Design review of the part built by this model. Coordinates are the model's own, in mm. A direction names the side the tool comes from. Coordinates: 2 decimals unless noted, no trailing zeros. Order: outer loops, then holes, each group sorted by start corner. A loop starts at its lowest first (then second) coordinate and runs counter-clockwise, first axis right, second up. Notation, with made-up numbers: (69, -19) -> (116, -19) arc R30 cw to (116, 11) -> close; hole circle Ø6 at (-26.75, 38.25). An arc over 180 degrees is marked (long way). Write item = value, one per line.
```python
from build123d import *

# Parameters (mm, degrees)
BASE_EXTRUDE_DEPTH = 3.5
SKETCH4_W          = 0.5
SKETCH4_H          = 10.618802154
CHAMFER_2_SIZE     = 0.64
FILLET_2_R         = 0.2


with BuildPart() as part:
    # Sketch1 → Base-Extrude (new body)
    with BuildSketch(Plane(origin=(0, 0, 0), x_dir=(0, 0, -1), z_dir=(1, 0, 0))):
        Polygon((4, 2.309401077), (4, -2.309401077), (0, -4.618802154), (-4, -2.309401077), (-4, 2.309401077), (0, 4.618802154), align=None)
    extrude(amount=BASE_EXTRUDE_DEPTH)

    # Sketch2 → Boss-Revolve1 (revolve)
    with BuildSketch(Plane.XY, mode=Mode.PRIVATE) as boss_revolve1_sk:
        Polygon((0, 0), (13.5, 0), (13.5, 1.8072), (13.5, 2.5), (0, 2.5), align=None)
    revolve(boss_revolve1_sk.sketch.rotate(Axis((0, 0, 0), (1, 0, 0)), 90), axis=Axis((0, 0, 0), (1, 0, 0)))

    # Sketch3 → Cut-Revolve1 (revolve, cut)
    with BuildSketch(Plane.XY):
        Polygon((0, 4), (3.244016936, 9.618802154), (3.244016936, 14.618802154), (-10, 14.618802154), (-10, 4), align=None)
    revolve(axis=Axis((0, 0, 0), (1, 0, 0)), mode=Mode.SUBTRACT)

    # Sketch5 → Cut-Revolve2 (revolve, cut)
    with BuildSketch(Plane.XY):
        Polygon((3.5, 4), (0.255983064, 9.618802154), (0.255983064, 14.618802154), (10.255983064, 14.618802154), (10.255983064, 4), align=None)
    revolve(axis=Axis((0, 0, 0), (1, 0, 0)), mode=Mode.SUBTRACT)

    # Sketch4 → Cut-Revolve3 (revolve, cut)
    with BuildSketch(Plane.XY, mode=Mode.PRIVATE) as cut_revolve3_sk:
        with Locations((3.25, 9.309401077)):
            Rectangle(SKETCH4_W, SKETCH4_H)
    revolve(cut_revolve3_sk.sketch.rotate(Axis((0, 0, 0), (1, 0, 0)), 270), axis=Axis((0, 0, 0), (1, 0, 0)), mode=Mode.SUBTRACT)

    # Chamfer 2
    chamfer_2_edges = [part.edges().sort_by_distance(p)[0] for p in [
        (13.5, 0, -2.5),
    ]]
    chamfer(chamfer_2_edges, length=CHAMFER_2_SIZE)

    # Fillet 2
    fillet_2_edges = [part.edges().sort_by_distance(p)[0] for p in [
        (3.5, 0, -2.5),
    ]]
    fillet(fillet_2_edges, radius=FILLET_2_R)


solid = part.part
```
(1) Insertion check: pin 1 (1.3 mm diameter, centred on y = 4.5, z = -1, fed in from +X); pin 2 (1.6 mm diameter, centred on y = 1, z = 3, fed in from +X); pin 3 (2 mm diameter, centred on y = -3, z = -1, fed in from +X); pin 4 (3 mm diameter, centred on y = -2.5, z = 1.5, fed in from +X). Each pin has a flat end and moves straight along its axis. Give the tip position at first contact, or say it passes through.
Report:
pin_1 = 3.5
pin_2 = 13
pin_3 = 13.2
pin_4 = 13.5
(2) For faces 1 (the cylindrical face through (3.254, -3.905, 0.867)), 2 (the flat face through (3, -2.1, 3.6)), 3 (the flat face through (3, -4.2, 0)), list the 3-axis set-ups (+Z, -Z, +X, -X, +Y, -Y) from which the entire face can be reached by the end or side of a thin tool; tool diameter is ignored.
Report:
face_1 = +X
face_2 = +Z, +X, -Y
face_3 = +X, -Y
(3) We need section A-A (x = 9.25). Write out the cut boundary in (y, z).
Report:
outline = circle Ø5 at (0, 0)
(4) For L1, parallel to Y at x = 10.5, z = 1.5; L2, parallel to X at y = 3.75, z = 1; L3, parallel to X at y = -2, z = -0.5, list the stretches that pass through material, from the lowest coordinate up.
Report:
L1 = -2 to 2
L2 = 0 to 3.5
L3 = 0 to 13.3
